Can you work these out from the model? Positions are in its coordinate system, mm. A direction names the side the tool comes from. Coordinates: 2 decimals unless noted, no trailing zeros. Order: outer loops, then holes, each group sorted by start corner. A loop starts at its lowest first (then second) coordinate and runs counter-clockwise, first axis right, second up. Notation, with made-up numbers: (51, -7.5) -> (95, -7.5) arc R29 cw to (95, 29.5) -> close; hole circle Ø11 at (34, -16.75). An arc over 180 degrees is marked (long way). Answer in a Markdown table with one row per item. Add a question column.
1. Imagine slicing it at B-B on y = 0. State how many separate pieces and enclosed holes the cut face has, plus the area to 3 significant figures.
2. On a 3-axis mill with a long thin cutter (end or side, diameter ignored), from which of +Z, -Z, +X, -X, +Y, -Y can I reach the whole of each face in a straight line? I mean faces 4 (the face through (-1, -25, 12)), 5 (the face through (19.567, -25.105, 5.916)). Say none if no direction works.
3. Will these pins go through, and if not, where does the flat tip stop? pin 1 (10 mm diameter, centred on x = 14, z = 25.5, fed in from -Y); pin 2 (6 mm diameter, centred on x = -15.5, z = 14, fed in from +Y); pin 3 (2 mm diameter, centred on y = -0.5, z = 15, fed in from -X); pin 4 (10 mm diameter, centred on x = 15.5, y = 12, fed in from -Z).
4. Imagine slicing it at C-C on z = 31.5. Write out the boundary of the cut face in (x, y).
5. If I drill on line 1 along X through (y, z) = (4, 11); line 2 along Y through (x, z) = (0, 32); line 3 along Y through (x, z) = (16.25, 7.5), over which ranges is the centre line in solid material (lowest first)? Write a range as [from, to].
6. Imagine slicing it at A-A on x = 0. Write out the boundary of the cut face in (y, z), plus the area to 3 significant figures.
7. We'd pull the mould along Y, two halves only. Please class faces 1 (the face through (-14.985, 0.66, 27.731)), 2 (the face through (-9, 9, 0)), 3 (the face through (-29.11, 26.7, 5.42)): pulls with the +Y half, pulls with the -Y half, needs draft (parallel to the pull), parting line crosses it, or undercut.
from build123d import *

# Parameters (mm, degrees)
SKETCH1_R           = 39.5
BOSS_EXTRUDE1_DEPTH = 12
SKETCH2_R           = 23.5
BOSS_EXTRUDE2_DEPTH = 33
SKETCH3_R           = 15
CUT_EXTRUDE1_DEPTH  = 35
SKETCH4_R           = 5.5
CUT_EXTRUDE2_DEPTH  = 3
SKETCH5_R           = 5.5
CUT_EXTRUDE3_DEPTH  = 7
CUT_EXTRUDE3_DRAFT  = 45
CHAMFER1_SIZE       = 1
SKETCH6_R           = 4.5
CUT_EXTRUDE4_DEPTH  = 21
FILLET1_R           = 1


with BuildPart() as part:
    # Sketch1 → Boss-Extrude1 (new body)
    with BuildSketch(Plane.XY):
        Circle(SKETCH1_R)
    extrude(amount=BOSS_EXTRUDE1_DEPTH)

    # Sketch2 → Boss-Extrude2 (add)
    with BuildSketch(Plane.XY.offset(12)):
        Circle(SKETCH2_R)
    extrude(amount=BOSS_EXTRUDE2_DEPTH)

    # Sketch3 → Cut-Extrude1 (cut)
    with BuildSketch(Plane.XY.offset(45)):
        Circle(SKETCH3_R)
    extrude(amount=-CUT_EXTRUDE1_DEPTH, mode=Mode.SUBTRACT)

    # Sketch4 → Cut-Extrude2 (cut)
    with BuildSketch(Plane.XY.offset(10)):
        Circle(SKETCH4_R)
    extrude(amount=-CUT_EXTRUDE2_DEPTH, mode=Mode.SUBTRACT)


with BuildPart() as cut_extrude3_tool:
    # Sketch5 → Cut-Extrude3 (with draft: the straight prism first)
    with BuildSketch(Plane.XY.offset(7)):
        Circle(SKETCH5_R)
    extrude(amount=-CUT_EXTRUDE3_DEPTH)
    # Cut-Extrude3: the draft: its side faces are tilted about the plane it starts from
    cut_extrude3_sides = [cut_extrude3_tool.faces().sort_by_distance(p)[0] for p in [
        (-5.5, 0, 3.5),
    ]]
    draft(cut_extrude3_sides, Plane.XY.offset(7), CUT_EXTRUDE3_DRAFT)


with BuildPart() as part_1:
    add(part.part)

    # Cut-Extrude3: cut by cut_extrude3_tool
    add(cut_extrude3_tool.part, mode=Mode.SUBTRACT)

    # Chamfer1
    chamfer1_edges = [part_1.edges().sort_by_distance(p)[0] for p in [
        (-15, 0, 45),
        (-39.5, 0, 12),
        (-23.5, 0, 45),
    ]]
    chamfer(chamfer1_edges, length=CHAMFER1_SIZE)

    # Sketch6 → Cut-Extrude4 (cut)
    with BuildSketch(Plane(origin=(0, 0, 0), x_dir=(-1, 0, 0), z_dir=(0, 0, -1))):
        with Locations((32.5, 0)):
            Circle(SKETCH6_R)
        with Locations((-16.25, -28.145825623)):
            Circle(SKETCH6_R)
        with Locations((-16.25, 28.145825623)):
            Circle(SKETCH6_R)
    extrude(amount=-CUT_EXTRUDE4_DEPTH, mode=Mode.SUBTRACT)

    # Fillet1
    fillet1_edges = [part_1.edges().sort_by_distance(p)[0] for p in [
        (-15, 0, 10),
        (-23.5, 0, 12),
    ]]
    fillet(fillet1_edges, radius=FILLET1_R)


solid = part_1.part
Answers follow:
| question | item | result |
|---|---|---|
| 1 | separate pieces | 3 |
| 1 | enclosed holes | 0 |
| 1 | area | 1,180 mm² |
| 2 | face 4 | +Z |
| 2 | face 5 | +Z, -Z |
| 3 | pin 1 | stops at y = -21.71 |
| 3 | pin 2 | stops at y = 36.56 |
| 3 | pin 3 | stops at x = -23.5 |
| 3 | pin 4 | stops at z = 0 |
| 4 | outline | circle Ø47 at (0, 0); hole circle Ø30 at (0, 0) |
| 5 | line 1 | x = [-39.3, -34.56], [-30.44, -14.46], [14.46, 39.3] |
| 5 | line 2 | y = [-23.5, -15], [15, 23.5] |
| 5 | line 3 | y = [-36, -32.65], [-23.65, 23.65], [32.65, 36] |
| 6 | outline | (-39.5, 0) -> (-12.5, 0) -> (-5.5, 7) -> (-5.5, 10) -> (-14, 10) arc R1 cw to (-15, 11) -> (-15, 44) -> (-16, 45) -> (-22.5, 45) -> (-23.5, 44) -> (-23.5, 13) arc R1 cw to (-24.5, 12) -> (-38.5, 12) -> (-39.5, 11) -> close; (5.5, 7) -> (12.5, 0) -> (39.5, 0) -> (39.5, 11) -> (38.5, 12) -> (24.5, 12) arc R1 cw to (23.5, 13) -> (23.5, 44) -> (22.5, 45) -> (16, 45) -> (15, 44) -> (15, 11) arc R1 cw to (14, 10) -> (5.5, 10) -> close |
| 6 | area | 1,290 mm² |
| 7 | face 1 | undercut |
| 7 | face 2 | needs draft |
| 7 | face 3 | parting line crosses it |
